from build123d import *

# Parameters (mm, degrees)
SKETCH1_R           = 100
SKETCH1_R_2         = 25.5
BOSS_EXTRUDE1_DEPTH = 80
FILLET1_R           = 5
CHAMFER1_SIZE       = 1


with BuildPart() as part:
    # Sketch1 → Boss-Extrude1 (new body)
    with BuildSketch(Plane.XY):
        Circle(SKETCH1_R)
        Circle(SKETCH1_R_2, mode=Mode.SUBTRACT)
    extrude(amount=BOSS_EXTRUDE1_DEPTH)

    # Fillet1
    fillet1_edges = [part.edges().sort_by_distance(p)[0] for p in [
        (-100, 0, 0),
        (-100, 0, 80),
    ]]
    fillet(fillet1_edges, radius=FILLET1_R)

    # Chamfer1
    chamfer1_edges = [part.edges().sort_by_distance(p)[0] for p in [
        (-25.5, 0, 0),
        (-25.5, 0, 80),
    ]]
    chamfer(chamfer1_edges, length=CHAMFER1_SIZE)


solid = part.part
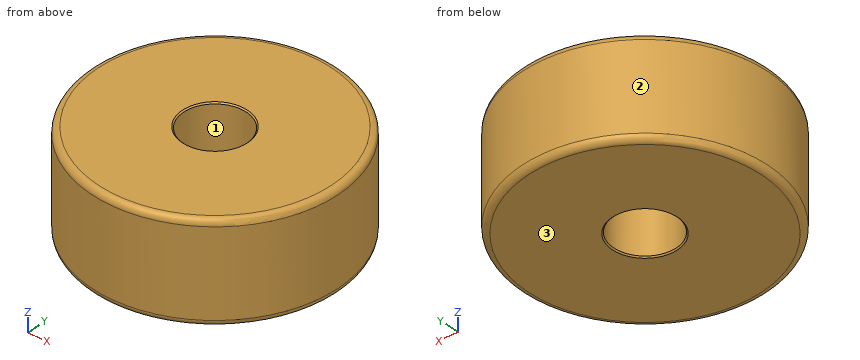
Part model, mm, in its own coordinate system. Face numbers are marked on the shaded views. Coordinates: 2 decimals unless noted, no trailing zeros. Order: outer loops, then holes, each group sorted by start corner. A loop starts at its lowest first (then second) coordinate and runs counter-clockwise, first axis right, second up. Notation, with made-up numbers: M -28,80 L 21,80 A18 cw 21,102 Z; hole C 76,54.25 d2. An arc over 180 degrees is marked long. One line per question, with ' | ' between items.
Q1. Two-plate mould, pull along X, no slides. Class the marked faces 1, 2 and 3: +X half, -X half, draft (parallel to the pull), parting line (faces both ways), or undercut.
A:
face 1: undercut | face 2: parting line | face 3: draft
Q2. Pin check, flat tips, straight feed: P1, Ø4, axis at x = -33.5, z = 12.5, coming from the -Y side; P2, Ø10, axis at x = 65.5, z = 54.5, coming from the -Y side; P3, Ø6, axis at x = -16, z = 9.5, coming from the -Y side. Stop position of each tip, or through.
A:
P1: stops at y = -94.91 | P2: stops at y = -79.62 | P3: stops at y = -99.15
Q3. Drill centre lines: line 1 (Y direction, x = 0, z = 18); line 2 (X direction, y = -14, z = 58.5). Where is each one in solid material? Low to high.
A:
line 1: y = -100 to -25.5, 25.5 to 100 | line 2: x = -99.02 to -21.31, 21.31 to 99.02
Q4. Slice it at C-C (z = 31). Give the cut face in (x, y), and give its area (3 significant figures).
A:
outline: C 0,0 d200; hole C 0,0 d51 | area: 29,400 mm^2
Q5. Slice it at A-A (x = 0). Give the cut face in (y, z), and give its area (3 significant figures).
A:
outline: M -100,5 A5 ccw -95,0 L -26.5,0 L -25.5,1 L -25.5,79 L -26.5,80 L -95,80 A5 ccw -100,75 Z; M 25.5,1 L 26.5,0 L 95,0 A5 ccw 100,5 L 100,75 A5 ccw 95,80 L 26.5,80 L 25.5,79 Z | area: 11,900 mm^2
